Part print with two shaded views. Sizes in mm from the minimum x, y, z corner. A direction names the side the tool comes from. Coordinates: 2 decimals unless noted, no trailing zeros. Write each loop counter-clockwise with the first axis right and the second up, starting at its lowest first coordinate (ties: lowest second). Pieces come first, ordered by that corner, then holes. Notation, with made-up numbers: M 28.25,-19 L 32.25,-19 A23 cw 32.25,9 Z; hole C -13,-31 d5. An arc over 180 degrees is marked long. One line per question, with ' | ' between items. Start each with the question number.
(1) Cut at D-D (y = 55.5). Write the cut outline in (x, z), plus the area to 3 significant figures.
(2) Flat gauge pins, fed straight in: pin 1 Ø5 at (x, z) = (48, 42.5) entering from -Y (1 decimal); pin 2 Ø2 at (x, y) = (105.5, 44.5) entering from -Z; pin 3 Ø13.5 at (y, z) = (6, 30) entering from -X; pin 4 Ø6 at (x, z) = (88.5, 19.5) entering from +Y. Where does each tip first touch, or does it go through?
(3) Cut at C-C (x = 54). Write the cut outline in (y, z), plus the area to 3 significant figures.
(4) Tool access for the marked faces 4, 5 and 6: list every direction of +Z, -Z, +X, -X, +Y, -Y with a clear straight run to the whole face (end or side of a thin tool).
(5) Cut at B-B (x = 104). Write the cut outline in (y, z).
(6) Cut at A-A (z = 39.5). Write the cut outline in (x, y).
(7) Wall check: probe 1 along X at (y, z) = (38.5, 39.5) (1 decimal); probe 2 along Z at (x, y) = (74, 56); probe 3 along Y at (x, z) = (104, 37.75). Give the ranges that are in metal, low to high.
(8) Two-plate mould, pull along Y, no slides. Class the marked faces 1, 2 and 3: +Y half, -Y half, draft (parallel to the pull), parting line (faces both ways), or undercut.
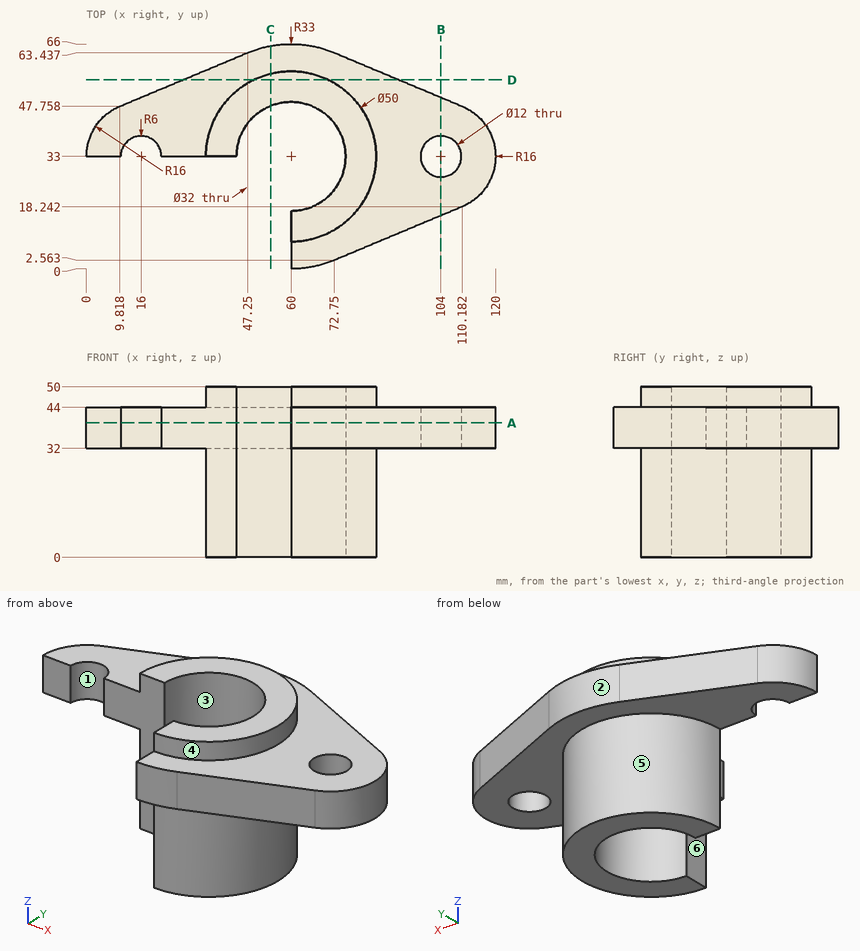
Filled in:
1) outline: M 28.3,32 L 49.1,32 L 49.1,0 L 70.9,0 L 70.9,32 L 91.7,32 L 91.7,44 L 70.9,44 L 70.9,50 L 49.1,50 L 49.1,44 L 28.3,44 Z | area: 1,590 mm²
2) pin 1: y = 39.8 | pin 2: z = 32 | pin 3: x = 60 | pin 4: through
3) outline: M 47.83,0 L 57.27,0 L 57.27,32 L 65.45,32 L 65.45,44 L 57.27,44 L 57.27,50 L 47.83,50 Z | area: 570 mm²
4) face 4: +Z | face 5: -Z | face 6: +Z, -Z, -X, -Y
5) outline: M 15.65,32 L 27,32 L 27,44 L 15.65,44 Z; M 39,32 L 50.35,32 L 50.35,44 L 39,44 Z
6) outline: M 0,33 L 10,33 A6 cw 22,33 L 44,33 A16 cw long 60,17 L 60,0 A33 ccw 72.75,2.56 L 110.18,18.24 A16 ccw 110.18,47.76 L 72.75,63.44 A33 ccw 47.25,63.44 L 9.82,47.76 A16 ccw Z; hole C 104,33 d12
7) probe 1: 1 to 13.6, 18.4 to 45, 75 to 101.6, 106.4 to 119 | probe 2: 32 to 44 | probe 3: 15.65 to 27, 39 to 50.35
8) face 1: -Y half | face 2: +Y half | face 3: undercut
